The listing builds one solid part. Answer for the finished solid, in the listing's coordinates (mm). A direction names the side the tool comes from. Coordinates: 2 decimals unless noted, no trailing zeros. Write each loop counter-clockwise with the first axis right and the second up, starting at its lowest first coordinate (ties: lowest second). Pieces come first, ordered by that corner, then holes.
```python
from build123d import *

# Parameters (mm, degrees)
EXTRUDE_1_DEPTH     = 740
SKETCH_2_R          = 3.5
CUT_EXTRUDE_1_DEPTH = 740
CUT_EXTRUDE_2_DEPTH = 740
SKETCH_4_R          = 6.5
CUT_EXTRUDE_3_DEPTH = 10


with BuildPart() as part:
    # 草图1 → 凸台-拉伸1 (new body)
    with BuildSketch(Plane.XY):
        with BuildLine():
            Line((0, 0), (25, 0))
            ThreePointArc((25, 0), (30.656854249, 2.343145751), (33, 8))
            Line((33, 8), (33, 35))
            ThreePointArc((33, 35), (34.464466094, 38.535533906), (38, 40))
            Line((38, 40), (928, 40))
            ThreePointArc((928, 40), (931.535533906, 38.535533906), (933, 35))
            Line((933, 35), (933, 8))
            ThreePointArc((933, 8), (935.343145751, 2.343145751), (941, 0))
            Line((941, 0), (966, 0))
            Line((966, 0), (966, 3))
            Line((966, 3), (941, 3))
            ThreePointArc((941, 3), (937.464466094, 4.464466094), (936, 8))
            Line((936, 8), (936, 35))
            ThreePointArc((936, 35), (933.656854249, 40.656854249), (928, 43))
            Line((928, 43), (38, 43))
            ThreePointArc((38, 43), (32.343145751, 40.656854249), (30, 35))
            Line((30, 35), (30, 8))
            ThreePointArc((30, 8), (28.535533906, 4.464466094), (25, 3))
            Line((25, 3), (0, 3))
            Line((0, 3), (0, 0))
        make_face()
    extrude(amount=EXTRUDE_1_DEPTH)

    # 草图2 → 切除-拉伸1 (cut)
    with BuildSketch(Plane(origin=(0, 43, 0), x_dir=(1, 0, 0), z_dir=(0, 1, 0))):
        with Locations(Location((78, -27.5, 0), (0, 0, 180))):
            Circle(SKETCH_2_R)
        with Locations(Location((483, -27.5, 0), (0, 0, 180))):
            Circle(SKETCH_2_R)
        with Locations(Location((888, -27.5, 0), (0, 0, 180))):
            Circle(SKETCH_2_R)
        with Locations(Location((78, -712.5, 0), (0, 0, 180))):
            Circle(SKETCH_2_R)
        with Locations(Location((888, -712.5, 0), (0, 0, 180))):
            Circle(SKETCH_2_R)
        with Locations(Location((483, -712.5, 0), (0, 0, 180))):
            Circle(SKETCH_2_R)
    extrude(amount=-CUT_EXTRUDE_1_DEPTH, mode=Mode.SUBTRACT)

    # 草图3 → 切除-拉伸2 (cut)
    with BuildSketch(Plane(origin=(0, 3, 0), x_dir=(1, 0, 0), z_dir=(0, 1, 0))):
        with BuildLine():
            Line((20.5, -22), (20.5, -28))
            ThreePointArc((20.5, -28), (16, -32.5), (11.5, -28))
            Line((11.5, -28), (11.5, -22))
            ThreePointArc((11.5, -22), (16, -17.5), (20.5, -22))
        make_face()
        with BuildLine():
            Line((20.5, -82), (20.5, -88))
            ThreePointArc((20.5, -88), (16, -92.5), (11.5, -88))
            Line((11.5, -88), (11.5, -82))
            ThreePointArc((11.5, -82), (16, -77.5), (20.5, -82))
        make_face()
        with BuildLine():
            Line((945.5, -82), (945.5, -88))
            ThreePointArc((945.5, -88), (950, -92.5), (954.5, -88))
            Line((954.5, -88), (954.5, -82))
            ThreePointArc((954.5, -82), (950, -77.5), (945.5, -82))
        make_face()
        with BuildLine():
            Line((945.5, -22), (945.5, -28))
            ThreePointArc((945.5, -28), (950, -32.5), (954.5, -28))
            Line((954.5, -28), (954.5, -22))
            ThreePointArc((954.5, -22), (950, -17.5), (945.5, -22))
        make_face()
        with BuildLine():
            Line((945.5, -658), (945.5, -652))
            ThreePointArc((945.5, -652), (950, -647.5), (954.5, -652))
            Line((954.5, -652), (954.5, -658))
            ThreePointArc((954.5, -658), (950, -662.5), (945.5, -658))
        make_face()
        with BuildLine():
            Line((945.5, -718), (945.5, -712))
            ThreePointArc((945.5, -712), (950, -707.5), (954.5, -712))
            Line((954.5, -712), (954.5, -718))
            ThreePointArc((954.5, -718), (950, -722.5), (945.5, -718))
        make_face()
        with BuildLine():
            Line((20.5, -658), (20.5, -652))
            ThreePointArc((20.5, -652), (16, -647.5), (11.5, -652))
            Line((11.5, -652), (11.5, -658))
            ThreePointArc((11.5, -658), (16, -662.5), (20.5, -658))
        make_face()
        with BuildLine():
            Line((20.5, -718), (20.5, -712))
            ThreePointArc((20.5, -712), (16, -707.5), (11.5, -712))
            Line((11.5, -712), (11.5, -718))
            ThreePointArc((11.5, -718), (16, -722.5), (20.5, -718))
        make_face()
    extrude(amount=-CUT_EXTRUDE_2_DEPTH, mode=Mode.SUBTRACT)

    # 草图4 → 切除-拉伸3 (cut)
    with BuildSketch(Plane(origin=(0, 43, 0), x_dir=(1, 0, 0), z_dir=(0, 1, 0))):
        with Locations(Location((483, -370, 0), (0, 0, 180))):
            Circle(SKETCH_4_R)
    extrude(amount=-CUT_EXTRUDE_3_DEPTH, mode=Mode.SUBTRACT)


solid = part.part
```
(1) Which of the six approach directions +Z, -Z, +X, -X, +Y, -Y give full straight-line access (tool end or side, diameter ignored) to faces 5 (the flat face through (33, 21, 365)), 6 (the flat face through (954, 3, 365)), 7 (the flat face through (13, 3, 365))?
(2) Section A-A, the plane z = 327 is taken. Write down the section's boundary in (x, y), plus the area to 3 significant figures.
(3) For a pull along X with two mould halves and no side action, classify faces 1 (the flat face through (933, 22, 365)), 2 (the flat face through (936, 21, 365)), 3 (the flat face through (953, 0, 365)), 4 (the flat face through (477, 40, 365)) as pulls with the +X half, pulls with the -X half, needs draft (parallel to the pull), parting line crosses it, or undercut.
(4) Find the intervals of material crossed by probe 1 along Z at (x, y) = (78, 42.15); probe 2 along X at (y, z) = (30, 227.5); probe 3 along X at (y, z) = (40.7, 712.5), in increasing order.
(5) Each of these flat-tipped pins is pushed along its axis until it touches: pin 1 (8 mm diameter, centred on y = 18.5, z = 153.5, fed in from -X); pin 2 (13.5 mm diameter, centred on y = 21, z = 399, fed in from +X); pin 3 (7.5 mm diameter, centred on x = 950.5, z = 389, fed in from +Y). Where does it stop, or does it pass through?
(6) Section B-B, the plane x = 794.5 is taken. Write down the section's boundary in (y, z), plus the area to 3 significant figures.
Solution:
1. face 5: +Z, -Z, -Y
1. face 6: +Z, -Z, +X, +Y
1. face 7: +Z, -Z, -X, +Y
2. outline: (0, 0) - (25, 0) arc R8 ccw to (33, 8) - (33, 35) arc R5 cw to (38, 40) - (928, 40) arc R5 cw to (933, 35) - (933, 8) arc R8 ccw to (941, 0) - (966, 0) - (966, 3) - (941, 3) arc R5 cw to (936, 8) - (936, 35) arc R8 ccw to (928, 43) - (38, 43) arc R8 ccw to (30, 35) - (30, 8) arc R5 cw to (25, 3) - (0, 3) - close
2. area: 3,100 mm2
3. face 1: undercut
3. face 2: pulls with the +X half
3. face 3: needs draft
3. face 4: undercut
4. probe 1: z = 0 to 24, 31 to 709, 716 to 740
4. probe 2: x = 30 to 33, 933 to 936
4. probe 3: x = 32.39 to 74.5, 81.5 to 479.5, 486.5 to 884.5, 891.5 to 933.61
5. pin 1: stops at x = 30
5. pin 2: stops at x = 936
5. pin 3: stops at y = 3
6. outline: (40, 0) - (43, 0) - (43, 740) - (40, 740) - close
6. area: 2,220 mm2
